For this review, take the finished solid that the model builds, in its own axes (mm). Coordinates: 2 decimals unless noted, no trailing zeros. Order: outer loops, then holes, each group sorted by start corner. A loop starts at its lowest first (then second) coordinate and runs counter-clockwise, first axis right, second up.
from build123d import *

# Parameters (mm, degrees)
BOSS_EXTRUDE1_DEPTH     = 5
CUT_EXTRUDE1_DEPTH      = 120.507321951
CUT_EXTRUDE1_DEPTH_BACK = 120.507321951
SKETCH2_R               = 5.5
CHAMFER1_SIZE           = 6


with BuildPart() as part:
    # Sketch1 → Boss-Extrude1 (new, symmetric)
    with BuildSketch(Plane.XY):
        with BuildLine():
            Line((-58, 96), (71, 96))
            Line((71, 96), (49.857864376, 74.857864376))
            ThreePointArc((49.857864376, 74.857864376), (45.52240935, 68.3693974), (44, 60.715728753))
            Line((44, 60.715728753), (44, -14))
            Line((44, -14), (-58, -14))
            Line((-58, -14), (-58, 96))
        make_face()
    extrude(amount=BOSS_EXTRUDE1_DEPTH, both=True)

    # Sketch2 → Cut-Extrude1 (cut, two sides: drawn at the far end of the back side and taken through both)
    with BuildSketch(Plane.XY.offset(-CUT_EXTRUDE1_DEPTH_BACK)):
        with Locations((-30, 0)):
            Circle(SKETCH2_R)
        with Locations((30, 0)):
            Circle(SKETCH2_R)
        with Locations((-45, 68)):
            Circle(SKETCH2_R)
        with Locations((30, 68)):
            Circle(SKETCH2_R)
    extrude(amount=CUT_EXTRUDE1_DEPTH + CUT_EXTRUDE1_DEPTH_BACK, mode=Mode.SUBTRACT)

    # Chamfer1
    chamfer1_edges = [part.edges().sort_by_distance(p)[0] for p in [
        (6.5, 96, -5),
    ]]
    chamfer(chamfer1_edges, length=CHAMFER1_SIZE)


solid = part.part
1. The part is to be moulded in two halves that separate along X. For faces 1 (the face through (44, 24, 0)), 2 (the face through (6, 93, -2)), 3 (the face through (-35.495, 0.242, -0.07)), say which applies: +X half, -X half, draft (parallel to the pull), parting line (faces both ways), or undercut.
Answer below:
face 1: +X half
face 2: draft
face 3: undercut
2. Take a section at C-C, the plane z = -2.25. Give the boundary of the cut face in (x, y), plus the area to 3 significant figures.
Answer below:
outline: (-58, -14) - (44, -14) - (44, 60.72) arc R20 cw to (49.86, 74.86) - (67.75, 92.75) - (-58, 92.75) - close; hole circle Ø11 at (-45, 68); hole circle Ø11 at (-30, 0); hole circle Ø11 at (30, 0); hole circle Ø11 at (30, 68)
area: 10,800 mm2
3. Clearance check with flat-ended pins moving along their axes: pin 1 Ø6.5 at (x, y) = (30, 68) entering from +Z; pin 2 Ø1 at (x, z) = (11.5, 0) entering from +Y; pin 3 Ø12.5 at (x, y) = (-45, 68) entering from -Z; pin 4 Ø1.5 at (y, z) = (53.5, 2.5) entering from +X. State where each tip first meets the part, or that it passes through.
Answer below:
pin 1: passes through
pin 2: stops at y = 95.5
pin 3: stops at z = -5
pin 4: stops at x = 44
4. Take a section at A-A, the plane x = -45. Give the boundary of the cut face in (y, z).
Answer below:
outline: (-14, -5) - (62.5, -5) - (62.5, 5) - (-14, 5) - close; (73.5, -5) - (90, -5) - (96, 1) - (96, 5) - (73.5, 5) - close
5. Take a section at D-D, the plane x = 30. Give the boundary of the cut face in (y, z), plus the area to 3 significant figures.
Answer below:
outline: (-14, -5) - (-5.5, -5) - (-5.5, 5) - (-14, 5) - close; (5.5, -5) - (62.5, -5) - (62.5, 5) - (5.5, 5) - close; (73.5, -5) - (90, -5) - (96, 1) - (96, 5) - (73.5, 5) - close
area: 862 mm2
6. Take a section at B-B, the plane y = 0. Give the boundary of the cut face in (x, z), plus the area to 3 significant figures.
Answer below:
outline: (-58, -5) - (-35.5, -5) - (-35.5, 5) - (-58, 5) - close; (-24.5, -5) - (24.5, -5) - (24.5, 5) - (-24.5, 5) - close; (35.5, -5) - (44, -5) - (44, 5) - (35.5, 5) - close
area: 800 mm2
7. To check wall thickness, follow L1, parallel to Y at x = 30, z = 1.5; L2, parallel to Y at x = 30, z = -3; L3, parallel to X at y = 0, z = 1.75. State the ranges of each line that lie inside material, in increasing order.
Answer below:
L1: y = -14 to -5.5, 5.5 to 62.5, 73.5 to 96
L2: y = -14 to -5.5, 5.5 to 62.5, 73.5 to 92
L3: x = -58 to -35.5, -24.5 to 24.5, 35.5 to 44
